Source: CAD feature listing. Evaluate the final solid. Frame: model axes, mm. Face numbers are marked on the shaded views. Coordinates: 2 decimals unless noted, no trailing zeros. Order: outer loops, then holes, each group sorted by start corner. A loop starts at its lowest first (then second) coordinate and runs counter-clockwise, first axis right, second up.
Item 1: Section A-A on y = 0. Return the cut outline in (x, z).
Item 2: Ray query, line 1 (Y direction, x = 0, z = -2); line 2 (X direction, y = 7.5, z = 6); line 3 (X direction, y = -1, z = 23.5). Return the intervals inside material, ascending.
Item 3: Mould query, pull axis Y, two halves, no side actions, for the marked faces 1 and 2. Classes: released by +Y, released by -Y, zero draft, split by the parting line, or undercut.
Item 4: Section C-C on z = -8. Return the cut outline in (x, y), then the cut area to 3 significant figures.
Item 5: Contact query for flat-ended pins moving along their axis: P1, Ø2, axis at x = 7, z = 14, coming from the +Y side; P2, Ø4, axis at x = 10, z = 11.5, coming from the -Y side; P3, Ø6, axis at y = 13, z = -17.5, coming from the -X side; P4, Ø3, axis at x = -9.5, y = 2.5, coming from the +Z side. Output: stop coordinate, or through.
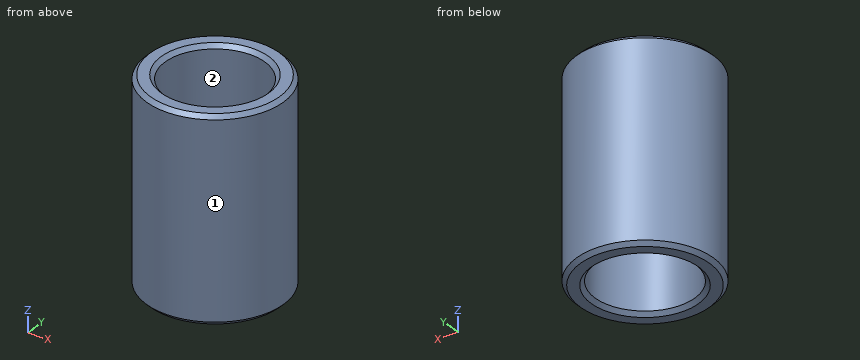
from build123d import *

# Parameters (mm, degrees)
SKETCH_1_R      = 17.5
SKETCH_1_R_2    = 12.75
EXTRUDE_1_DEPTH = 25.5
CHAMFER_1_SIZE  = 1


with BuildPart() as part:
    # 草图1 → 凸台-拉伸1 (new, symmetric)
    with BuildSketch(Plane.XY):
        Circle(SKETCH_1_R)
        Circle(SKETCH_1_R_2, mode=Mode.SUBTRACT)
    extrude(amount=EXTRUDE_1_DEPTH, both=True)

    # 倒角1
    chamfer_1_edges = [part.edges().sort_by_distance(p)[0] for p in [
        (-17.5, 0, -25.5),
        (-17.5, 0, 25.5),
        (-12.75, 0, -25.5),
        (-12.75, 0, 25.5),
    ]]
    chamfer(chamfer_1_edges, length=CHAMFER_1_SIZE)


solid = part.part
Answer list:
1. outline: (-17.5, -24.5) - (-16.5, -25.5) - (-13.75, -25.5) - (-12.75, -24.5) - (-12.75, 24.5) - (-13.75, 25.5) - (-16.5, 25.5) - (-17.5, 24.5) - close; (12.75, -24.5) - (13.75, -25.5) - (16.5, -25.5) - (17.5, -24.5) - (17.5, 24.5) - (16.5, 25.5) - (13.75, 25.5) - (12.75, 24.5) - close
2. line 1: y = -17.5 to -12.75, 12.75 to 17.5
2. line 2: x = -15.81 to -10.31, 10.31 to 15.81
2. line 3: x = -17.47 to -12.71, 12.71 to 17.47
3. face 1: split by the parting line
3. face 2: undercut
4. outline: circle Ø35 at (0, 0); hole circle Ø25.5 at (0, 0)
4. area: 451 mm2
5. P1: stops at y = 16.44
5. P2: stops at y = -15.56
5. P3: stops at x = -14.36
5. P4: passes through
